```python
from build123d import *

# Parameters (mm, degrees)
SKETCH1_W                                         = 9
SKETCH1_H                                         = 14
BOSS_EXTRUDE1_DEPTH                               = 12.5
CUT_EXTRUDE1_DEPTH                                = 3
SKETCH3_W                                         = 9
SKETCH3_H                                         = 10
BOSS_EXTRUDE2_DEPTH                               = 2
FILLET1_R                                         = 1
HOLE_SIZE_PER_HEX_SOCKET_SCREW_TYPE_1_D           = 3.4
HOLE_SIZE_PER_HEX_SOCKET_SCREW_TYPE_1_CBORE_D     = 6
HOLE_SIZE_PER_HEX_SOCKET_SCREW_TYPE_1_CBORE_DEPTH = 3.4


with BuildPart() as part:
    # Sketch1 → Boss-Extrude1 (new body)
    with BuildSketch(Plane(origin=(0, 0, 0), x_dir=(1, 0, 0), z_dir=(0, 1, 0))):
        Rectangle(SKETCH1_W, SKETCH1_H)
    extrude(amount=BOSS_EXTRUDE1_DEPTH)

    # Sketch2 → Cut-Extrude1 (cut)
    with BuildSketch(Plane.XZ):
        with BuildLine():
            Line((1, 1), (-2, 1))
            ThreePointArc((-2, 1), (-3, -1), (-2, -3))
            Line((-2, -3), (1, -3))
            ThreePointArc((1, -3), (2, -1), (1, 1))
        make_face()
    extrude(amount=-CUT_EXTRUDE1_DEPTH, mode=Mode.SUBTRACT)

    # Sketch3 → Boss-Extrude2 (add)
    with BuildSketch(Plane.XY.offset(7)):
        with Locations((0, 17.5)):
            Rectangle(SKETCH3_W, SKETCH3_H)
    extrude(amount=-BOSS_EXTRUDE2_DEPTH)

    # Fillet1
    fillet1_edges = [part.edges().sort_by_distance(p)[0] for p in [
        (0, 22.5, 5),
    ]]
    fillet(fillet1_edges, radius=FILLET1_R)

    # Hole size (per hex socket screw type) 1 (through all)
    with Locations(Plane(origin=(-0.5, 12.5, -1), x_dir=(0, 0, 1), z_dir=(0, 1, 0))):
        with Locations((0, 0)):
            CounterBoreHole(HOLE_SIZE_PER_HEX_SOCKET_SCREW_TYPE_1_D / 2, HOLE_SIZE_PER_HEX_SOCKET_SCREW_TYPE_1_CBORE_D / 2, HOLE_SIZE_PER_HEX_SOCKET_SCREW_TYPE_1_CBORE_DEPTH)


solid = part.part
```
Can you work these out from the model? Positions are in its coordinate system, mm. A direction names the side the tool comes from. Give positions to 0.01 mm unless a question says otherwise; leave off trailing zeros. Loops run counter-clockwise (first coordinate to the right, second up) from the corner with the lowest first, then second, coordinate; pieces in that order, holes last. Notation, with made-up numbers: M -17.5,52 L -2.5,52 A23 ccw -2.5,90 Z; hole C 13,-23 d7. An arc over 180 degrees is marked long. One line per item, written item: value.
(1) Suppose I cut it at A-A on z = -1. List the corners of the cut face in (x, y) for me, plus the area to 3 significant figures.
Returned:
outline: M -4.5,0 L -3,0 L -3,3 L -2.2,3 L -2.2,9.1 L -3.5,9.1 L -3.5,12.5 L -4.5,12.5 Z; M 1.2,3 L 2,3 L 2,0 L 4.5,0 L 4.5,12.5 L 2.5,12.5 L 2.5,9.1 L 1.2,9.1 Z
area: 56.4 mm^2
(2) Suppose I cut it at B-B on x = -0.5. List the corners of the cut face in (y, z) for me, plus the area to 3 significant figures.
Returned:
outline: M 0,-7 L 12.5,-7 L 12.5,-4 L 9.1,-4 L 9.1,-2.7 L 3,-2.7 L 3,-3 L 0,-3 Z; M 0,1 L 3,1 L 3,0.7 L 9.1,0.7 L 9.1,2 L 12.5,2 L 12.5,5 L 21.5,5 A1 ccw 22.5,6 L 22.5,7 L 0,7 Z
area: 142 mm^2
(3) Which directions (+Z, -Z, +X, -X, +Y, -Y) give clear straight access to the entire face, cutting with the end or side of a thin tool? Please do faces 1 (the face through (0.933, 6.007, -1.914)), 2 (the face through (0, 9.1, 1)), 3 (the face through (1, 12.5, -4)), 4 (the face through (2, 1, -1)), 5 (the face through (-0.1, 0, 1.5)).
Returned:
face 1: +Y, -Y
face 2: +Y
face 3: -Z, +X, -X, +Y
face 4: -Y
face 5: +Z, -Z, +X, -X, -Y
(4) Will these pins go through, and if not, where does the flat tip stop? pin 1 (2.5 mm diameter, centred on x = -1, y = 18, fed in from -Z); pin 2 (1 mm diameter, centred on y = 14, z = 1, fed in from +X); pin 3 (4 mm diameter, centred on x = -2, z = 1, fed in from +Y); pin 4 (2.5 mm diameter, centred on x = -2, z = -1, fed in from +Y).
Returned:
pin 1: z = 5
pin 2: through
pin 3: y = 12.5
pin 4: y = 9.1
(5) Suppose I cut it at D-D on x = 3. List the corners of the cut face in (y, z) for me.
Returned:
outline: M 0,-7 L 12.5,-7 L 12.5,5 L 21.5,5 A1 ccw 22.5,6 L 22.5,7 L 0,7 Z
(6) Suppose I cut it at C-C on y = 10. List the corners of the cut face in (x, z) for me, plus the area to 3 significant figures.
Returned:
outline: M -4.5,-7 L 4.5,-7 L 4.5,7 L -4.5,7 Z; hole C -0.5,-1 d6
area: 97.7 mm^2
(7) I need wall thicknesses on line 1 (X direction, y = 11.4, z = -1); line 2 (Z direction, x = -0.5, y = 1.75); line 3 (Z direction, x = 1.5, y = 21.25). Which ranges of each line are inside material? Lowest first, please.
Returned:
line 1: -4.5 to -3.5, 2.5 to 4.5
line 2: -7 to -3, 1 to 7
line 3: 5 to 7
